from build123d import *

# Parameters (mm, degrees)
SKETCH_1_R               = 5
SKETCH_1_R_2             = 6
EXTRUDE_1_DEPTH          = 10
SKETCH_2_R               = 6
CUT_EXTRUDE_1_DEPTH      = 10
SKETCH_3_R               = 8
SKETCH_3_R_2             = 4
EXTRUDE_2_DEPTH          = 10
CUT_EXTRUDE_3_DEPTH      = 417.865256367
CUT_EXTRUDE_3_DEPTH_BACK = 10
SKETCH_4_R               = 5
SKETCH_5_R               = 5
EXTRUDE_3_DEPTH          = 10
SKETCH_6_R               = 5
EXTRUDE_4_DEPTH          = 10
EXTRUDE_5_DEPTH          = 10


with BuildPart() as part:
    # 草图1 → 凸台-拉伸1 (new body)
    with BuildSketch(Plane.XY):
        with BuildLine():
            Line((-200.997267146, -87.263605576), (110, -87.263605576))
            Line((110, -87.263605576), (110, 0))
            Line((110, 0), (110, 79.983892276))
            Line((110, 79.983892276), (85.070632456, 79.983892276))
            Line((85.070632456, 79.983892276), (85.070632456, 49.983892276))
            ThreePointArc((85.070632456, 49.983892276), (55.070632456, 19.983892276), (25.070632456, 49.983892276))
            Line((25.070632456, 49.983892276), (25.070632456, 79.983892276))
            Line((25.070632456, 79.983892276), (10.070632456, 79.983892276))
            Line((10.070632456, 79.983892276), (10.070632456, 166.983892276))
            Line((10.070632456, 166.983892276), (-15.514893523, 166.983892276))
            Line((-15.514893523, 166.983892276), (-15.514893523, 127.416711183))
            ThreePointArc((-15.514893523, 127.416711183), (-55.514893523, 87.416711183), (-95.514893523, 127.416711183))
            Line((-95.514893523, 127.416711183), (-95.514893523, 232.416711183))
            Line((-95.514893523, 232.416711183), (-86.514893523, 232.416711183))
            Line((-86.514893523, 232.416711183), (-86.514893523, 332.416711183))
            Line((-86.514893523, 332.416711183), (-110.997267146, 332.416711183))
            Line((-110.997267146, 332.416711183), (-110.997267146, 302.681550212))
            ThreePointArc((-110.997267146, 302.681550212), (-140.997267146, 272.681550212), (-170.997267146, 302.681550212))
            Line((-170.997267146, 302.681550212), (-170.997267146, 332.681550212))
            Line((-170.997267146, 332.681550212), (-200.997267146, 332.681550212))
            Line((-200.997267146, 332.681550212), (-250.997267146, 332.681550212))
            Line((-250.997267146, 332.681550212), (-250.997267146, 212.681550212))
            Line((-250.997267146, 212.681550212), (-250.997267146, 207.681550212))
            Line((-250.997267146, 207.681550212), (-200.997267146, 207.681550212))
            Line((-200.997267146, 207.681550212), (-200.997267146, 182.681550212))
            Line((-200.997267146, 182.681550212), (-200.997267146, -44.649528276))
            Line((-200.997267146, -44.649528276), (-200.997267146, -87.263605576))
        make_face()
        with Locations((96.070632456, 49.983892276)):
            Circle(SKETCH_1_R, mode=Mode.SUBTRACT)
        with Locations((14.070632456, 49.983892276)):
            Circle(SKETCH_1_R, mode=Mode.SUBTRACT)
        with Locations((-3.014893523, 127.416711183)):
            Circle(SKETCH_1_R_2, mode=Mode.SUBTRACT)
        with Locations((-108.014893523, 127.416711183)):
            Circle(SKETCH_1_R_2, mode=Mode.SUBTRACT)
        with Locations((-99.997267146, 302.681550212)):
            Circle(SKETCH_1_R, mode=Mode.SUBTRACT)
        with Locations((-181.997266842, 302.67655009)):
            Circle(SKETCH_1_R, mode=Mode.SUBTRACT)
        with Locations((-37.523881476, 10.659198545)):
            Circle(SKETCH_1_R_2, mode=Mode.SUBTRACT)
        with Locations((-92.336608934, -13.745000039)):
            Circle(SKETCH_1_R_2, mode=Mode.SUBTRACT)
        with Locations((-147.149336393, -38.149198624)):
            Circle(SKETCH_1_R_2, mode=Mode.SUBTRACT)
        with Locations((-235.997267146, 222.681550212)):
            Circle(SKETCH_1_R_2, mode=Mode.SUBTRACT)
        with Locations((-195.999464127, 222.681550212)):
            Circle(SKETCH_1_R_2, mode=Mode.SUBTRACT)
        with Locations((-235.997267146, 252.681550212)):
            Circle(SKETCH_1_R_2, mode=Mode.SUBTRACT)
        with Locations((-195.997267146, 252.681550131)):
            Circle(SKETCH_1_R_2, mode=Mode.SUBTRACT)
    extrude(amount=EXTRUDE_1_DEPTH)

    # 草图2 → 切除-拉伸1 (cut)
    with BuildSketch(Plane.XY.offset(10)):
        with Locations((-158.358654267, 28.055066971)):
            Circle(SKETCH_2_R)
        with Locations((-187.336429056, 35.819638324)):
            Circle(SKETCH_2_R)
    extrude(amount=-CUT_EXTRUDE_1_DEPTH, mode=Mode.SUBTRACT)

    # 草图3 → 凸台-拉伸2 (add)
    with BuildSketch(Plane.XY.offset(10)):
        with BuildLine():
            Line((110, -87.263605576), (62, -87.263605576))
            Line((62, -87.263605576), (44.5, -87.263605576))
            Line((44.5, -87.263605576), (44.5, -112.263605576))
            ThreePointArc((44.5, -112.263605576), (57, -124.763605576), (69.5, -112.263605576))
            Line((69.5, -112.263605576), (69.5, -102.263605576))
            Line((69.5, -102.263605576), (240, -102.263605576))
            Line((240, -102.263605576), (240, -87.263605576))
            Line((240, -87.263605576), (110, -87.263605576))
        make_face()
        with Locations((57, -112.263605576)):
            Circle(SKETCH_3_R, mode=Mode.SUBTRACT)
        with Locations((225, -94.763605576)):
            Circle(SKETCH_3_R_2, mode=Mode.SUBTRACT)
        with Locations((205, -94.763605576)):
            Circle(SKETCH_3_R_2, mode=Mode.SUBTRACT)
    extrude(amount=-EXTRUDE_2_DEPTH)

    # 草图4 → 切除-拉伸3 (cut, two sides: drawn at the far end of the back side and taken through both)
    # profile 1 of 2: a face of its own
    with BuildSketch(Plane(origin=(0, 0, 0), x_dir=(-1, 0, 0), z_dir=(0, 0, -1)).offset(-CUT_EXTRUDE_3_DEPTH_BACK)):
        with BuildLine():
            ThreePointArc((170.997267146, 302.681550212), (162.210470582, 281.468346776), (140.997267146, 272.681550212))
            Line((140.997267146, 272.681550212), (250.997267146, 272.681550212))
            Line((250.997267146, 272.681550212), (250.997267146, 332.681550212))
            Line((250.997267146, 332.681550212), (170.997267146, 332.681550212))
            Line((170.997267146, 332.681550212), (170.997267146, 302.681550212))
        make_face()
        with Locations((181.997266842, 302.67655009)):
            Circle(SKETCH_4_R, mode=Mode.SUBTRACT)
    # profile 2 of 2: a face of its own
    with BuildSketch(Plane(origin=(0, 0, 0), x_dir=(-1, 0, 0), z_dir=(0, 0, -1)).offset(-CUT_EXTRUDE_3_DEPTH_BACK)):
        with BuildLine():
            Line((86.514893523, 272.681550212), (140.997267146, 272.681550212))
            ThreePointArc((140.997267146, 272.681550212), (119.784063711, 281.468346776), (110.997267146, 302.681550212))
            Line((110.997267146, 302.681550212), (110.997267146, 332.416711183))
            Line((110.997267146, 332.416711183), (86.514893523, 332.416711183))
            Line((86.514893523, 332.416711183), (86.514893523, 272.681550212))
        make_face()
        with Locations((99.997267146, 302.681550212)):
            Circle(SKETCH_4_R, mode=Mode.SUBTRACT)
    extrude(amount=CUT_EXTRUDE_3_DEPTH + CUT_EXTRUDE_3_DEPTH_BACK, mode=Mode.SUBTRACT)

    # 草图5 → 凸台-拉伸3 (add)
    with BuildSketch(Plane(origin=(0, 0, 0), x_dir=(-1, 0, 0), z_dir=(0, 0, -1))):
        with Locations((-96.070632456, 49.983892276)):
            Circle(SKETCH_5_R)
    extrude(amount=-EXTRUDE_3_DEPTH)

    # 草图6 → 凸台-拉伸4 (add)
    with BuildSketch(Plane(origin=(0, 0, 0), x_dir=(-1, 0, 0), z_dir=(0, 0, -1))):
        with Locations((-14.070632456, 49.983892276)):
            Circle(SKETCH_6_R)
    extrude(amount=-EXTRUDE_4_DEPTH)

    # 草图7 → 凸台-拉伸5 (add)
    with BuildSketch(Plane(origin=(0, 0, 0), x_dir=(-1, 0, 0), z_dir=(0, 0, -1))):
        with BuildLine():
            Line((-85.070632456, 79.983892276), (-85.070632456, 49.983892276))
            ThreePointArc((-85.070632456, 49.983892276), (-55.070632456, 19.983892276), (-25.070632456, 49.983892276))
            Line((-25.070632456, 49.983892276), (-25.070632456, 79.983892276))
            Line((-25.070632456, 79.983892276), (-85.070632456, 79.983892276))
        make_face()
    extrude(amount=-EXTRUDE_5_DEPTH)


solid = part.part
Work out the finished part from the listing and answer in its coordinate system (mm). A direction names the side the tool comes from. Coordinates: 2 decimals unless noted, no trailing zeros. Order: outer loops, then holes, each group sorted by start corner. A loop starts at its lowest first (then second) coordinate and runs counter-clockwise, first axis right, second up. Notation, with made-up numbers: (78, -14.5) - (83, -14.5) arc R12 cw to (83, -8.5) - close; hole circle Ø6 at (26, -5.75). An arc over 180 degrees is marked (long way). Put each result on its own line as item: value. Start each with the question number.
1) Find the intervals of material crossed by line 1 (X direction, y = 11, z = 4.75); line 2 (X direction, y = 154.5, z = 8.5); line 3 (X direction, y = 123.5, z = 2.5), in increasing order. Write a range as from..to.
2) Flat-ended cylindrical pins translate along their axes: pin 1 (5 mm diameter, centred on y = -4.5, z = 5.5, fed in from +X); pin 2 (1 mm diameter, centred on x = 170.5, z = 2, fed in from +Y); pin 3 (3 mm diameter, centred on x = -129, z = 4, fed in from -Y); pin 4 (11 mm diameter, centred on x = -108.01, y = 127.42, fed in from -Z). Find the tip coordinate at first contact, or state that the pin passes through.
3) Find section C-C (z = 8.25). State how many separate pieces and enclosed holes the cut face has, plus the area to 3 significant figures.
4) Find section D-D (x = -132). Give the vertices of the cut face in (y, z).
5) For faces 1 (the cylindrical face through (-54.635, 87.426, 4.93)), 2 (the flat face through (-226, 207.682, 5)), 3 (the flat face through (110, -5, 5)), determine the directions among +Z, -Z, +X, -X, +Y, -Y from which every point of the face is accessible in a straight line to the end or side of a thin tool.
6) Find section B-B (y = 114.5). Give the vertices of the cut face in (x, z).
7) For a pull along X with two mould halves and no side action, classify faces 4 (the flat face through (176, -87.264, 5)), 5 (the flat face through (-15.515, 147, 5)), 6 (the cylindrical face through (56.73, -124.76, 5.07)) as released by +X, released by -X, zero draft, split by the parting line, or undercut.
8) Find section A-A (x = 57). Give the vertices of the cut face in (y, z), plus the area to 3 significant figures.
Results list:
1. line 1: x = -201..-43.51, -31.53..110
1. line 2: x = -201..-95.51, -15.51..10.07
1. line 3: x = -201..-112.56, -103.47..-95.32, -15.71..-7.56, 1.53..10.07
2. pin 1: stops at x = 110
2. pin 2: stops at y = -87.26
2. pin 3: stops at y = -87.26
2. pin 4: passes through
3. separate pieces: 1
3. enclosed holes: 14
3. area: 81,300 mm^2
4. outline: (-87.26, 0) - (272.68, 0) - (272.68, 10) - (-87.26, 10) - close
5. face 1: +Z, -Z
5. face 2: +Z, -Z, -X, -Y
5. face 3: +Z, -Z, +X, +Y
6. outline: (-201, 0) - (-93.37, 0) - (-93.37, 10) - (-201, 10) - close; (-17.66, 0) - (10.07, 0) - (10.07, 10) - (-17.66, 10) - close
7. face 4: zero draft
7. face 5: undercut
7. face 6: split by the parting line
8. outline: (-124.76, 0) - (-120.26, 0) - (-120.26, 10) - (-124.76, 10) - close; (-104.26, 0) - (79.98, 0) - (79.98, 10) - (-104.26, 10) - close
8. area: 1,890 mm^2
